Source: CAD feature listing. Evaluate the final solid. Frame: model axes, mm. A direction names the side the tool comes from. Give positions to 0.01 mm unless a question says otherwise; leave off trailing zeros. Loops run counter-clockwise (first coordinate to the right, second up) from the corner with the lowest first, then second, coordinate; pieces in that order, holes last. Notation, with made-up numbers: (53, 43) - (85, 43) arc R27 cw to (85, 61) - close; hole circle Ø9 at (-29.75, 63). An arc over 180 degrees is marked (long way). Put each result on its own line as item: value.
```python
from build123d import *

# Parameters (mm, degrees)
BOSS_EXTRUDE1_DEPTH = 10
CHAMFER1_SIZE       = 1
CUT_EXTRUDE1_START  = 4.754218
SKETCH3_R           = 3.5
CUT_EXTRUDE1_DEPTH  = 20
SKETCH7_R           = 11.1
CUT_EXTRUDE2_DEPTH  = 20


with BuildPart() as part:
    # Sketch1 → Boss-Extrude1 (new body)
    with BuildSketch(Plane(origin=(0, 0, 0), x_dir=(1, 0, 0), z_dir=(0, 1, 0))):
        with BuildLine():
            Line((9.923855052, 12.745782203), (-9.923855052, 12.745782203))
            ThreePointArc((-9.923855052, 12.745782203), (-15.7379694, 10.992816749), (-19.614159094, 6.318207995))
            ThreePointArc((-19.614159094, 6.318207995), (-21.768533293, 3.720074961), (-25, 2.745782203))
            Line((-25, 2.745782203), (-32, 2.745782203))
            Line((-32, 2.745782203), (-32, -12.254217797))
            Line((-32, -12.254217797), (-22.930291583, -12.254217797))
            ThreePointArc((-22.930291583, -12.254217797), (-16.191557905, -13.687244076), (-10.619046633, -17.738319737))
            ThreePointArc((-10.619046633, -17.738319737), (0, -22.468623982), (10.619046633, -17.738319737))
            ThreePointArc((10.619046633, -17.738319737), (16.191557905, -13.687244076), (22.930291583, -12.254217797))
            Line((22.930291583, -12.254217797), (32, -12.254217797))
            Line((32, -12.254217797), (32, 2.745782203))
            Line((32, 2.745782203), (25, 2.745782203))
            ThreePointArc((25, 2.745782203), (21.768533293, 3.720074961), (19.614159094, 6.318207995))
            ThreePointArc((19.614159094, 6.318207995), (15.7379694, 10.992816749), (9.923855052, 12.745782203))
        make_face()
    extrude(amount=BOSS_EXTRUDE1_DEPTH)

    # Chamfer1
    chamfer1_edges = [part.edges().sort_by_distance(p)[0] for p in [
        (32, 5, -2.745782203),
        (32, 5, 12.254217797),
        (-32, 5, 12.254217797),
        (-32, 5, -2.745782203),
    ]]
    chamfer(chamfer1_edges, length=CHAMFER1_SIZE)

    # Sketch3 → Cut-Extrude1 (cut)
    with BuildSketch(Plane.XY.offset(CUT_EXTRUDE1_START)):
        with Locations((27.40080015, 5)):
            Circle(SKETCH3_R)
        with Locations(Location((-27.40080015, 5, 0), (0, 0, 180))):
            Circle(SKETCH3_R)
    extrude(amount=CUT_EXTRUDE1_DEPTH, mode=Mode.SUBTRACT)

    # Sketch7 → Cut-Extrude2 (cut)
    with BuildSketch(Plane(origin=(0, 10, 0), x_dir=(1, 0, 0), z_dir=(0, 1, 0))):
        with Locations(Location((0, -4.754217797, 0), (0, 0, 180))):
            Circle(SKETCH7_R)
    extrude(amount=-CUT_EXTRUDE2_DEPTH, mode=Mode.SUBTRACT)


solid = part.part
```
1) Section query B-B, the plane z = 6. Output: boundary loops of the cut face in (x, y).
Check result:
outline: (-32, 0) - (-11.03, 0) - (-11.03, 10) - (-32, 10) - close; (11.03, 0) - (32, 0) - (32, 10) - (11.03, 10) - close; hole circle Ø7 at (-27.4, 5); hole circle Ø7 at (27.4, 5)
2) Section query A-A, the plane x = 0. Output: boundary loops of the cut face in (y, z), plus the area to 3 significant figures.
Check result:
outline: (0, -12.75) - (10, -12.75) - (10, -6.35) - (0, -6.35) - close; (0, 15.85) - (10, 15.85) - (10, 22.47) - (0, 22.47) - close
area: 130 mm²
3) Section query D-D, the plane z = -4. Output: boundary loops of the cut face in (x, y).
Check result:
outline: (-21.38, 0) - (-6.82, 0) - (-6.82, 10) - (-21.38, 10) - close; (6.82, 0) - (21.38, 0) - (21.38, 10) - (6.82, 10) - close
4) Pin query (flat end, axial travel): P1, Ø1.5, axis at y = 3, z = -4.5, coming from the +X side; P2, Ø5, axis at y = 5.5, z = -7.5, coming from the +X side; P3, Ø4, axis at x = 27, y = 7, coming from the +Z side. Return the tip coordinate at first contact, or that it passes through.
Check result:
P1: x = 21.72
P2: x = 20.39
P3: z = 12.25
5) Mould query, pull axis X, two halves, no side actions, for faces 1 (the flat face through (-32, 5, 5)), 2 (the cylindrical face through (-30.74, 3.95, 8.45)), 3 (the flat face through (32, 5, 5)). Classes: pulls with the +X half, pulls with the -X half, needs draft (parallel to the pull), parting line crosses it, or undercut.
Check result:
face 1: pulls with the -X half
face 2: undercut
face 3: pulls with the +X half
6) Material intervals for line 1 along X through (y, z) = (6, 10.5); line 2 along X through (y, z) = (5, 8.5); line 3 along Z through (x, y) = (0, 1.75), sorted ascending. Write a range as [from, to].
Check result:
line 1: [-32, -30.75], [-24.05, -9.5], [9.5, 24.05], [30.75, 32]
line 2: [-32, -30.9], [-23.9, -10.45], [10.45, 23.9], [30.9, 32]
line 3: [-12.75, -6.35], [15.85, 22.47]
7) Access query for faces 4 (the flat face through (-27, 5, 4.754)), 5 (the flat face through (-28, 5, -2.746)), 6 (the flat face through (23.3, 4.9, 12.254)). Directions: +Z, -Z, +X, -X, +Y, -Y. A direction counts if a zero-diameter tool reaches every point of the face in a straight line with its end or side. Return the directions, or none.
Check result:
face 4: +Z
face 5: -Z, -X, +Y, -Y
face 6: +Z, +X, +Y, -Y
8) Section query C-C, the plane y = 5. Output: boundary loops of the cut face in (x, z) (3 decimals), plus the area to 3 significant figures.
Check result:
outline: (-32, -1.746) - (-31, -2.746) - (-25, -2.746) arc R5.846 cw to (-19.614, -6.318) arc R10.518 ccw to (-9.924, -12.746) - (9.924, -12.746) arc R10.518 ccw to (19.614, -6.318) arc R5.846 cw to (25, -2.746) - (31, -2.746) - (32, -1.746) - (32, 11.254) - (31, 12.254) - (30.901, 12.254) - (30.901, 4.754) - (23.901, 4.754) - (23.901, 12.254) - (22.93, 12.254) arc R16.561 cw to (10.619, 17.738) arc R14.284 ccw to (-10.619, 17.738) arc R16.561 cw to (-22.93, 12.254) - (-23.901, 12.254) - (-23.901, 4.754) - (-30.901, 4.754) - (-30.901, 12.254) - (-31, 12.254) - (-32, 11.254) - close; hole circle Ø22.2 at (0, 4.754)
area: 1,060 mm²
